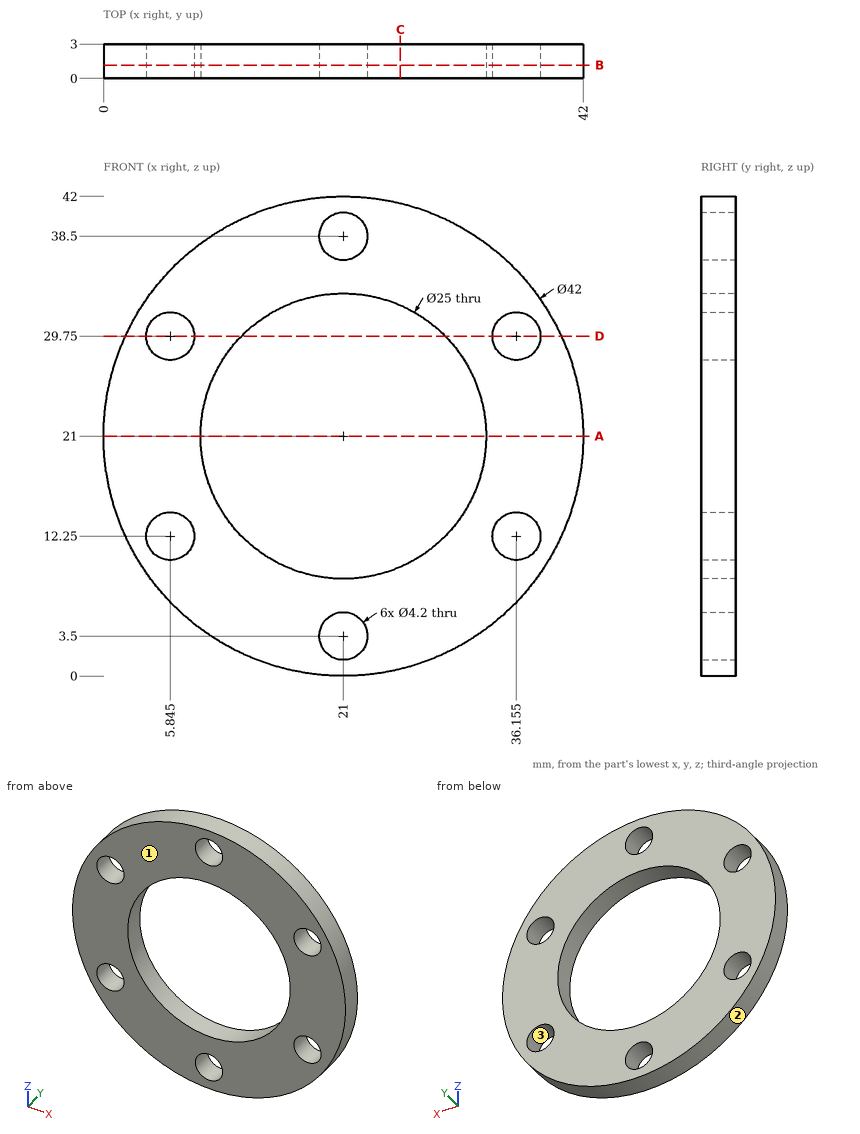
The drawing under review shows one solid part. Ordinate dimensions are in mm from its lowest x, y, z. Round coordinates to 2 decimals unless told otherwise and drop trailing zeros. Write each loop counter-clockwise with the first axis right and the second up, starting at its lowest first coordinate (ties: lowest second). Pieces come first, ordered by that corner, then holes. Notation, with made-up numbers: (-4.75, 83) -> (13.25, 83) arc R29 cw to (13.25, 117) -> close; hole circle Ø11 at (-40, 52.5). An arc over 180 degrees is marked (long way). Put each result on its own line as item: value.
Q1. Consider section D-D on z = 29.75. State the section outline as (x, y) points (1 decimal).
Determined:
outline: (1.9, 0) -> (3.7, 0) -> (3.7, 3) -> (1.9, 3) -> close; (7.9, 0) -> (12.1, 0) -> (12.1, 3) -> (7.9, 3) -> close; (29.9, 0) -> (34.1, 0) -> (34.1, 3) -> (29.9, 3) -> close; (38.3, 0) -> (40.1, 0) -> (40.1, 3) -> (38.3, 3) -> close
Q2. The part is to be moulded in two halves that separate along Z. For the marked faces 1, 2 and 3, say which applies: released by +Z, released by -Z, zero draft, split by the parting line, or undercut.
Determined:
face 1: zero draft
face 2: split by the parting line
face 3: undercut
Q3. To check wall thickness, follow L1, parallel to X at y = 1.8, z = 21; L2, parallel to X at y = 0.9, z = 29.75 (1 decimal); L3, parallel to X at y = 1.3, z = 28 (1 decimal). State the ranges of each line that lie inside material, in increasing order. Write a range as [from, to].
Determined:
L1: x = [0, 8.5], [33.5, 42]
L2: x = [1.9, 3.7], [7.9, 12.1], [29.9, 34.1], [38.3, 40.1]
L3: x = [1.2, 4.7], [7, 10.6], [31.4, 35], [37.3, 40.8]
Q4. Consider section A-A on z = 21. State the section outline as (x, y) points, and give its area (3 significant figures).
Determined:
outline: (0, 0) -> (8.5, 0) -> (8.5, 3) -> (0, 3) -> close; (33.5, 0) -> (42, 0) -> (42, 3) -> (33.5, 3) -> close
area: 51.0 mm^2
Q5. Clearance check with a flat-ended pin moving along its axis: pin 1 Ø1.5 at (x, y) = (16, 2) entering from -Z (1 decimal). State where the tip first meets the part, or that it passes through.
Determined:
pin 1: stops at z = 0.4
Q6. Consider section C-C on x = 26. State the section outline as (y, z) points.
Determined:
outline: (0, 0.6) -> (3, 0.6) -> (3, 9.54) -> (0, 9.54) -> close; (0, 32.46) -> (3, 32.46) -> (3, 41.4) -> (0, 41.4) -> close
Q7. Consider section B-B on y = 1.15. Give the number of separate pieces and of enclosed holes in the cut face.
Determined:
separate pieces: 1
enclosed holes: 7
